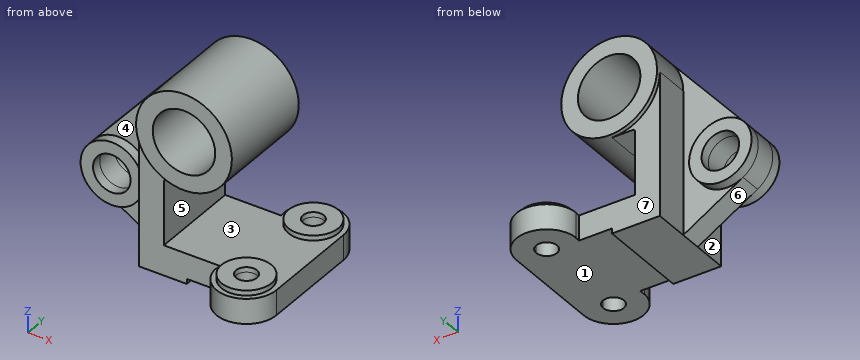
```python
from build123d import *

# Parameters (mm, degrees)
BASE_PROFILE_SKETCH_R     = 12.5
BASE_BODY_DEPTH           = 15
BOSS_PAD_SKETCH_R         = 30
BOSS_PAD_6MM_DEPTH        = 6
BORE_SKETCH_R             = 12.5
BORE_CUT_DEPTH            = 145.976722269
ARM_BLOCK_SKETCH_R        = 57.5
ARM_BLOCK_SKETCH_R_2      = 37.5
ARM_BLOCK_DEPTH           = 60
WEB_DEPTH                 = 55
WEB_POCKET_SKETCH_W       = 39.351063387
WEB_POCKET_SKETCH_H       = 7.1816736
WEB_POCKET_SKETCH_W_2     = 45.776165888
WEB_POCKET_SKETCH_H_2     = 5.709571084
WEB_POCKET_CUT_DEPTH      = 97
MOUNTING_PLATE_SKETCH_R   = 37.5
MOUNTING_PLATE_SKETCH_R_2 = 22.5
MOUNTING_PLATE_DEPTH      = 25
LUG_BOSSES_DEPTH          = 13
LUG_HOLES_SKETCH_R        = 22.5
LUG_HOLES_CUT_DEPTH       = 329.05411139


with BuildPart() as part:
    # Base Profile Sketch → Base Body (new, symmetric)
    with BuildSketch(Plane.XY):
        with BuildLine():
            Line((-36, -60), (-102.5, -60))
            Line((-102.5, -60), (-102.5, 60))
            Line((-102.5, 60), (-36, 60))
            ThreePointArc((-36, 60), (0, 96), (36, 60))
            Line((36, 60), (36, -60))
            ThreePointArc((36, -60), (0, -96), (-36, -60))
        make_face()
        with Locations((0, 60)):
            Circle(BASE_PROFILE_SKETCH_R, mode=Mode.SUBTRACT)
        with Locations((0, -60)):
            Circle(BASE_PROFILE_SKETCH_R, mode=Mode.SUBTRACT)
    extrude(amount=BASE_BODY_DEPTH, both=True)

    # Boss Pad Sketch → Boss Pad 6mm (add)
    with BuildSketch(Plane.XY.offset(15)):
        with Locations((0, -60)):
            Circle(BOSS_PAD_SKETCH_R)
        with Locations((0, 60)):
            Circle(BOSS_PAD_SKETCH_R)
    extrude(amount=BOSS_PAD_6MM_DEPTH)

    # Bore Sketch → Bore Cut (cut, through all)
    with BuildSketch(Plane(origin=(0, 0, -15), x_dir=(-1, 0, 0), z_dir=(0, 0, -1))):
        with Locations((0, -60)):
            Circle(BORE_SKETCH_R)
        with Locations((0, 60)):
            Circle(BORE_SKETCH_R)
    extrude(amount=-BORE_CUT_DEPTH, mode=Mode.SUBTRACT)



with BuildPart() as body_2:
    # Arm Block Sketch → Arm Block (new, symmetric)
    with BuildSketch(Plane(origin=(0, 0, 0), x_dir=(1, 0, 0), z_dir=(0, 1, 0))):
        with Locations(Location((-75, -151, 0), (0, 0, 270))):
            Circle(ARM_BLOCK_SKETCH_R)
        with Locations(Location((-75, -151, 0), (0, 0, 270))):
            Circle(ARM_BLOCK_SKETCH_R_2, mode=Mode.SUBTRACT)
    extrude(amount=ARM_BLOCK_DEPTH, both=True)


with BuildPart() as part_1:
    add(part.part)

    add(body_2.part)  # Web merges body 2
    # Web Profile Sketch → Web (add, symmetric)
    with BuildSketch(Plane(origin=(0, 0, 0), x_dir=(1, 0, 0), z_dir=(0, 1, 0))):
        with BuildLine():
            Line((-132.5, -151), (-132.5, 21))
            Line((-132.5, 21), (-75, 21))
            Line((-75, 21), (-75, 15))
            Line((-75, 15), (-36, 15))
            Line((-36, 15), (-36, -15))
            Line((-36, -15), (-102.5, -15))
            Line((-102.5, -15), (-102.5, -91.5))
            ThreePointArc((-102.5, -91.5), (-101.914213562, -92.914213562), (-100.5, -93.5))
            Line((-100.5, -93.5), (-75, -93.5))
            ThreePointArc((-75, -93.5), (-115.658639918, -110.341360082), (-132.5, -151))
        make_face()
    extrude(amount=WEB_DEPTH, both=True)

    # Web Pocket Sketch → Web Pocket Cut (cut)
    with BuildSketch(Plane.ZY.offset(132.5)):
        with Locations((-1.324468307, -58.5908368)):
            Rectangle(WEB_POCKET_SKETCH_W, WEB_POCKET_SKETCH_H)
        with Locations((1.888082944, 57.854785542)):
            Rectangle(WEB_POCKET_SKETCH_W_2, WEB_POCKET_SKETCH_H_2)
    extrude(amount=-WEB_POCKET_CUT_DEPTH, mode=Mode.SUBTRACT)



with BuildPart() as body_2_2:
    # Mounting Plate Sketch → Mounting Plate (new, symmetric)
    with BuildSketch(Plane(origin=(0, 0, 0), x_dir=(1, 0, 0), z_dir=(0, 1, 0))):
        with Locations(Location((-185, -54, 0), (0, 0, 270))):
            Circle(MOUNTING_PLATE_SKETCH_R)
        with Locations(Location((-185, -54, 0), (0, 0, 270))):
            Circle(MOUNTING_PLATE_SKETCH_R_2, mode=Mode.SUBTRACT)
    extrude(amount=MOUNTING_PLATE_DEPTH, both=True)


with BuildPart() as part_2:
    add(part_1.part)

    add(body_2_2.part)  # Lug Bosses merges body 2 2
    # Lug Bosses Sketch → Lug Bosses (add, symmetric)
    with BuildSketch(Plane(origin=(0, 0, 0), x_dir=(1, 0, 0), z_dir=(0, 1, 0))):
        with BuildLine():
            Line((-132.5, 21), (-204.216934712, -21.798145701))
            ThreePointArc((-204.216934712, -21.798145701), (-222.016718342, -47.998953157), (-213.406251821, -78.481316498))
            Line((-213.406251821, -78.481316498), (-118.556252792, -188.53801863))
            Line((-118.556252792, -188.53801863), (-118.556252792, 21))
            Line((-118.556252792, 21), (-132.5, 21))
        make_face()
    extrude(amount=LUG_BOSSES_DEPTH, both=True)

    # Lug Holes Sketch → Lug Holes Cut (cut, through all)
    with BuildSketch(Plane.XZ.offset(25)):
        with Locations(Location((-185, 54, 0), (0, 0, 90))):
            Circle(LUG_HOLES_SKETCH_R)
    extrude(amount=-LUG_HOLES_CUT_DEPTH, mode=Mode.SUBTRACT)


solid = part_2.part
```
Geometry: final body of the model. Coordinates: model frame, mm. Face numbers are marked on the shaded views. A direction names the side the tool comes from. Round coordinates to 2 decimals unless told otherwise and drop trailing zeros. Write each loop counter-clockwise with the first axis right and the second up, starting at its lowest first coordinate (ties: lowest second). Pieces come first, ordered by that corner, then holes.
Item 1: Material intervals for L1, parallel to X at y = 21.75, z = 54; L2, parallel to Z at x = -185, y = 21.25; L3, parallel to X at y = -29, z = 151, sorted ascending.
Item 2: Section query D-D (y = 69). Return loops of the section in (x, z), plus the area to 3 significant figures.
Item 3: Set-up query: the marked faces 1, 2, 3 and 4. Return all of +Z, -Z, +X, -X, +Y, -Y with unobstructed straight access to the full face (end or side cutting, diameter ignored); none if empty.
Item 4: Section query B-B (z = 54). Return loops of the section in (x, y).
Item 5: Pin query (flat end, axial travel): P1, Ø10, axis at y = 36, z = 156.5, coming from the +X side; P2, Ø1.5, axis at x = -127.5, y = 21.5, coming from the +Z side; P3, Ø8, axis at y = 2.5, z = 131, coming from the -X side. Return the tip coordinate at first contact, or that it passes through.
Item 6: Mould query, pull axis Z, two halves, no side actions, for the marked faces 5, 6 and 7. Classes: +Z half, -Z half, draft (parallel to the pull), parting line (faces both ways), or undercut.
Item 7: Section query C-C (x = 0). Return loops of the section in (y, z), plus the area to 3 significant figures.
Item 8: Section query A-A (y = -17). Return loops of the section in (x, z).
Completed:
1. L1: x = -222.5 to -207.5, -162.5 to -147.5, -132.5 to -102.5
1. L2: z = 16.5 to 31.5, 76.5 to 91.5
1. L3: x = -132.5 to -112.5, -37.5 to -17.5
2. outline: (-34.86, -15) - (-8.67, -15) - (-8.67, 21) - (-28.62, 21) - (-28.62, 15) - (-34.86, 15) - close; (8.67, -15) - (34.86, -15) - (34.86, 15) - (28.62, 15) - (28.62, 21) - (8.67, 21) - close
2. area: 1,810 mm2
3. face 1: -Z, +X, +Y, -Y
3. face 2: +Z, -Z, -Y
3. face 3: none
3. face 4: -Y
4. outline: (-222.5, -25) - (-207.5, -25) - (-207.5, 25) - (-222.5, 25) - close; (-162.5, -25) - (-147.5, -25) - (-147.5, -13) - (-132.5, -13) - (-132.5, -55) - (-102.5, -55) - (-102.5, 55) - (-132.5, 55) - (-132.5, 13) - (-147.5, 13) - (-147.5, 25) - (-162.5, 25) - close
5. P1: stops at x = -17.5
5. P2: stops at z = 176.06
5. P3: stops at x = -171.59
6. face 5: undercut
6. face 6: -Z half
6. face 7: draft
7. outline: (-96, -15) - (-72.5, -15) - (-72.5, 21) - (-90, 21) - (-90, 15) - (-96, 15) - close; (-47.5, -15) - (47.5, -15) - (47.5, 21) - (30, 21) - (30, 15) - (-30, 15) - (-30, 21) - (-47.5, 21) - close; (72.5, -15) - (96, -15) - (96, 15) - (90, 15) - (90, 21) - (72.5, 21) - close
7. area: 4,680 mm2
8. outline: circle Ø75 at (-185, 54); (-132.5, -21) - (-75, -21) - (-75, -15) - (36, -15) - (36, 15) - (-102.5, 15) - (-102.5, 91.5) arc R2 cw to (-100.5, 93.5) - (-75, 93.5) arc R57.5 ccw (long way) to (-132.5, 151) - close; hole circle Ø45 at (-185, 54); hole circle Ø75 at (-75, 151)
